from build123d import *

# Parameters (mm, degrees)
BASE_BODY_DEPTH         = 100
MOUNTING_FLANGE_DEPTH   = 15
FLANGE_HOLES_CUT_DEPTH  = 15
FLANGE_NOTCH_PROFILE_R  = 5
FLANGE_NOTCH_CUT_DEPTH  = 15
HOUSING_BLOCK_DEPTH     = 39.5
HOUSING_RECESS_DEPTH    = 22
PIVOT_BOSS_DEPTH        = 45
SIDE_PIN_HOLE_PROFILE_R = 10
SIDE_PIN_HOLE_DEPTH     = 17.5
PIVOT_BORE_PROFILE_R    = 5
PIVOT_BORE_DEPTH        = 30
BEARING_HOUSING_DEPTH   = 22
BEARING_BORE_DEPTH      = 40


with BuildPart() as part:
    # Base Body Profile → Base Body (new body)
    with BuildSketch(Plane.XY):
        with BuildLine():
            Line((0, 0), (0, 90))
            Line((0, 90), (25, 90))
            ThreePointArc((25, 90), (26.464466094, 86.464466094), (30, 85))
            Line((30, 85), (30, 5))
            ThreePointArc((30, 5), (26.464466094, 3.535533906), (25, 0))
            Line((25, 0), (0, 0))
        make_face()
    extrude(amount=BASE_BODY_DEPTH)

    # Mounting Flange Profile → Mounting Flange (add)
    with BuildSketch(Plane(origin=(0, 0, 0), x_dir=(-1, 0, 0), z_dir=(0, 0, -1))):
        with BuildLine():
            Line((-130, 45), (-130, 75))
            ThreePointArc((-130, 75), (-127.071067812, 82.071067812), (-120, 85))
            Line((-120, 85), (-30, 85))
            Line((-30, 85), (-30, 5))
            Line((-30, 5), (-120, 5))
            ThreePointArc((-120, 5), (-127.071067812, 7.928932188), (-130, 15))
            Line((-130, 15), (-130, 45))
        make_face()
    extrude(amount=-MOUNTING_FLANGE_DEPTH)

    # Flange Holes Profile → Flange Holes Cut (cut)
    with BuildSketch(Plane(origin=(0, 0, 0), x_dir=(-1, 0, 0), z_dir=(0, 0, -1))):
        with BuildLine():
            Line((-130, 60), (-130, 30))
            Line((-130, 30), (-105, 30))
            Line((-105, 30), (-105, 33))
            ThreePointArc((-105, 33), (-93, 45), (-105, 57))
            Line((-105, 57), (-105, 60))
            Line((-105, 60), (-130, 60))
        make_face()
    extrude(amount=-FLANGE_HOLES_CUT_DEPTH, mode=Mode.SUBTRACT)

    # Flange Notch Profile → Flange Notch Cut (cut)
    with BuildSketch(Plane.XY.offset(15)):
        with Locations((120, 75)):
            Circle(FLANGE_NOTCH_PROFILE_R)
        with Locations((120, 15)):
            Circle(FLANGE_NOTCH_PROFILE_R)
    extrude(amount=-FLANGE_NOTCH_CUT_DEPTH, mode=Mode.SUBTRACT)

    # Housing Block Profile → Housing Block (add)
    with BuildSketch(Plane.XY.offset(100)):
        with BuildLine():
            Line((30, 85), (88.457666717, 63.123682675))
            ThreePointArc((88.457666717, 63.123682675), (100, 45), (88.457666717, 26.876317325))
            Line((88.457666717, 26.876317325), (30, 5))
            Line((30, 5), (30, 85))
        make_face()
    extrude(amount=-HOUSING_BLOCK_DEPTH)

    # Housing Recess Profile → Housing Recess (cut)
    with BuildSketch(Plane.XY.offset(100)):
        with BuildLine():
            Line((30, 85), (30, 5))
            Line((30, 5), (88.457666717, 26.876317325))
            ThreePointArc((88.457666717, 26.876317325), (100, 45), (88.457666717, 63.123682675))
            Line((88.457666717, 63.123682675), (30, 85))
        make_face()
    extrude(amount=-HOUSING_RECESS_DEPTH, mode=Mode.SUBTRACT)

    # Pivot Boss Profile → Pivot Boss (add)
    with BuildSketch(Plane.XY.offset(15)):
        Polygon((70, 70.031002054), (30, 85), (30, 45), (70, 45), align=None)
        Polygon((70, 45), (30, 45), (30, 5), (70, 22.19323305), align=None)
    extrude(amount=PIVOT_BOSS_DEPTH)

    # Side Pin Hole Profile → Side Pin Hole (cut)
    with BuildSketch(Plane.XY.offset(78)):
        with Locations((80, 45)):
            Circle(SIDE_PIN_HOLE_PROFILE_R)
    extrude(amount=-SIDE_PIN_HOLE_DEPTH, mode=Mode.SUBTRACT)

    # Pivot Bore Profile → Pivot Bore (cut)
    with BuildSketch(Plane(origin=(70, 0, 0), x_dir=(0, 0, -1), z_dir=(1, 0, 0))):
        with Locations((-37.5, 45)):
            Circle(PIVOT_BORE_PROFILE_R)
    extrude(amount=-PIVOT_BORE_DEPTH, mode=Mode.SUBTRACT)

    # Bearing Housing Profile → Bearing Housing (add)
    with BuildSketch(Plane.XY.offset(100)):
        with BuildLine():
            ThreePointArc((30, 5), (70, 45), (30, 85))
            Line((30, 85), (30, 75))
            ThreePointArc((30, 75), (60, 45), (30, 15))
            Line((30, 15), (30, 5))
        make_face()
    extrude(amount=-BEARING_HOUSING_DEPTH)

    # Bearing Bore Profile → Bearing Bore (cut)
    with BuildSketch(Plane.XY.offset(100)):
        with BuildLine():
            Line((30, 75), (10, 75))
            Line((10, 75), (10, 65))
            Line((10, 65), (0, 65))
            Line((0, 65), (0, 25))
            Line((0, 25), (10, 25))
            Line((10, 25), (10, 15))
            Line((10, 15), (30, 15))
            ThreePointArc((30, 15), (60, 45), (30, 75))
        make_face()
    extrude(amount=-BEARING_BORE_DEPTH, mode=Mode.SUBTRACT)


solid = part.part
Verification items for the finished model (mm, model axes). A direction names the side the tool comes from. Coordinates: 2 decimals unless noted, no trailing zeros. Order: outer loops, then holes, each group sorted by start corner. A loop starts at its lowest first (then second) coordinate and runs counter-clockwise, first axis right, second up. Notation, with made-up numbers: M -39.5,-35.75 L 0.5,-35.75 A22 cw 0.5,-3.75 Z; hole C 20,35 d6. An arc over 180 degrees is marked long. One line per item, written item: value. Start each with the question number.
Item 1: Access from +Z, -Z, +X, -X, +Y, -Y to the whole of each face (thin tool, end or side, straight path). Record for faces 5 (the flat face through (105, 31, 7)), 6 (the cylindrical face through (59.993, 45.66, 80.526)), 7 (the flat face through (74, 5, 7)), 8 (the flat face through (35, 46, 60)), 9 (the flat face through (49.72, 13.476, 37.185)).
Item 2: Sectioned sample at D-D (y = 53). Enter the section's corners in (x, z).
Item 3: Gauge pin test, flat ends, axial feed: pin 1 (16.5 mm diameter, centred on x = 59, z = 4.5, fed in from -Y); pin 2 (8 mm diameter, centred on x = 120, y = 75, fed in from +Z); pin 3 (1.5 mm diameter, centred on y = 32.5, z = 81.5, fed in from +X); pin 4 (6 mm diameter, centred on y = 52, z = 36, fed in from +X). Record the tip position at first contact, or that the pin passes through.
Item 4: Sectioned sample at C-C (z = 87). Enter the section's corners in (x, y).
Item 5: Scan lines: probe 1 along Y at (x, z) = (120, 7.25); probe 2 along Z at (x, y) = (61, 60); probe 3 along Z at (x, y) = (66, 46). Record each from-to range of solid material in increasing order.
Item 6: Mould release check, pull along Z, two halves, no side actions. Record for faces 1 (the flat face through (56, 62, 100)), 2 (the cylindrical face through (55.21, 48.379, 41.185)), 3 (the flat face through (65, 45, 60.5)), 4 (the cylindrical face through (124.619, 13.085, 7.605)): released by +Z, released by -Z, zero draft, split by the parting line, or undercut.
Item 7: Sectioned sample at A-A (z = 74). Enter the section's corners in (x, y).
Item 8: Sectioned sample at B-B (x = 80). Enter the section's corners in (y, z).
Conclusion:
1. face 5: +Z, -Z, +X
1. face 6: +Z
1. face 7: +Z, -Z, +X, -Y
1. face 8: +X
1. face 9: +X, -Y
2. outline: M 0,0 L 96.06,0 L 96.06,15 L 70,15 L 70,60 L 0,60 Z; M 58.91,60.5 L 74,60.5 L 74,78 L 69.19,78 L 69.19,100 L 58.91,100 Z; M 86,60.5 L 98.33,60.5 L 98.33,78 L 86,78 Z
3. pin 1: stops at y = 5
3. pin 2: passes through
3. pin 3: stops at x = 68.24
3. pin 4: stops at x = 70
4. outline: M 0,0 L 25,0 A5 cw 30,5 A40 ccw 30,85 A5 cw 25,90 L 0,90 L 0,65 L 10,65 L 10,75 L 30,75 A30 cw 30,15 L 10,15 L 10,25 L 0,25 Z
5. probe 1: y = 5 to 10, 20 to 30, 60 to 70, 80 to 85
5. probe 2: z = 0 to 60, 60.5 to 100
5. probe 3: z = 0 to 32.6, 42.4 to 60, 60.5 to 100
6. face 1: released by +Z
6. face 2: undercut
6. face 3: undercut
6. face 4: zero draft
7. outline: M 0,0 L 25,0 A5 cw 30,5 L 88.46,26.88 A20 ccw 88.46,63.12 L 30,85 A5 cw 25,90 L 0,90 L 0,65 L 10,65 L 10,75 L 30,75 A30 cw 30,15 L 10,15 L 10,25 L 0,25 Z; hole C 80,45 d20
8. outline: M 5,0 L 85,0 L 85,15 L 5,15 Z; M 23.71,60.5 L 35,60.5 L 35,78 L 23.71,78 Z; M 55,60.5 L 66.29,60.5 L 66.29,78 L 55,78 Z
